Design review of the part built by this model. Coordinates are the model's own, in mm. Face numbers are marked on the shaded views. A direction names the side the tool comes from. Coordinates: 2 decimals unless noted, no trailing zeros. Write each loop counter-clockwise with the first axis right and the second up, starting at its lowest first coordinate (ties: lowest second). Pieces come first, ordered by that corner, then holes.
Q1. Take a section at A-A, the plane x = 62.5. Write out the cut boundary in (y, z), plus the area to 3 significant figures.
Q2. Take a section at C-C, the plane x = 99.5. Write out the cut boundary in (y, z).
Q3. For L1, parallel to Z at x = 62, y = 4; L2, parallel to X at y = 6, z = 50; L3, parallel to Z at x = 74, y = 45, list the stretches that pass through material, from the lowest coordinate up.
Q4. For the marked faces 1 and 2, list the 3-axis set-ups (+Z, -Z, +X, -X, +Y, -Y) from which the entire face can be reached by the end or side of a thin tool; tool diameter is ignored.
Q5. Take a section at B-B, the plane z = 50. Write out the cut boundary in (x, y), plus the area to 3 significant figures.
Q6. The part is to be moulded in two halves that separate along Z. For the marked faces 3, 4 and 5, say which applies: released by +Z, released by -Z, zero draft, split by the parting line, or undercut.
Q7. Take a section at D-D, the plane y = 26.5. Write out the cut boundary in (x, z), plus the area to 4 significant figures.
Q8. For pin 1 Ø8 at (x, z) = (36, 54) entering from +Y, flat-tipped, find the tip position at first contact; note if it passes through.
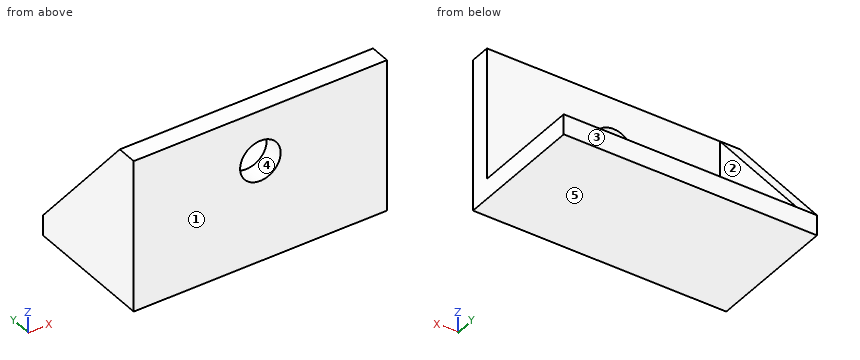
from build123d import *

# Parameters (mm, degrees)
BASE_PLATE_PROFILE_W  = 125
BASE_PLATE_PROFILE_H  = 10
BASE_PLATE_DEPTH      = 75
BACK_WALL_PROFILE_W   = 125
BACK_WALL_PROFILE_H   = 10
BACK_WALL_DEPTH       = 55
END_WALL_PROFILE_W    = 10
END_WALL_PROFILE_H    = 65
END_WALL_DEPTH        = 55
GUSSET_TRIM_CUT_DEPTH = 55
BASE_HOLE_20_SKETCH_R = 10
BASE_HOLE_20_DEPTH    = 55


with BuildPart() as part:
    # Base Plate Profile → Base Plate (new body)
    with BuildSketch(Plane.XY):
        with Locations((62.5, 5)):
            Rectangle(BASE_PLATE_PROFILE_W, BASE_PLATE_PROFILE_H)
    extrude(amount=BASE_PLATE_DEPTH)

    # Back Wall Profile → Back Wall (add)
    with BuildSketch(Plane(origin=(0, 10, 0), x_dir=(1, 0, 0), z_dir=(0, 1, 0))):
        with Locations((62.5, -5)):
            Rectangle(BACK_WALL_PROFILE_W, BACK_WALL_PROFILE_H)
    extrude(amount=BACK_WALL_DEPTH)

    # End Wall Profile → End Wall (add)
    with BuildSketch(Plane(origin=(0, 10, 0), x_dir=(1, 0, 0), z_dir=(0, 1, 0))):
        with Locations((5, -42.5)):
            Rectangle(END_WALL_PROFILE_W, END_WALL_PROFILE_H)
    extrude(amount=END_WALL_DEPTH)

    # Gusset Trim Profile → Gusset Trim Cut (cut)
    with BuildSketch(Plane(origin=(10, 0, 0), x_dir=(0, 0, -1), z_dir=(1, 0, 0))):
        Polygon((-10, 65), (-75, 10), (-75, 65), align=None)
    extrude(amount=-GUSSET_TRIM_CUT_DEPTH, mode=Mode.SUBTRACT)

    # Base Hole Ø20 Sketch → Base Hole Ø20 (cut)
    with BuildSketch(Plane(origin=(0, 10, 0), x_dir=(1, 0, 0), z_dir=(0, 1, 0))):
        with Locations(Location((62.5, -50, 0), (0, 0, 270))):
            Circle(BASE_HOLE_20_SKETCH_R)
    extrude(amount=-BASE_HOLE_20_DEPTH, mode=Mode.SUBTRACT)


solid = part.part
Responses:
1. outline: (0, 0) - (65, 0) - (65, 10) - (10, 10) - (10, 40) - (0, 40) - close; (0, 60) - (10, 60) - (10, 75) - (0, 75) - close
1. area: 1,100 mm2
2. outline: (0, 0) - (65, 0) - (65, 10) - (10, 10) - (10, 75) - (0, 75) - close
3. L1: z = 0 to 40.01, 59.99 to 75
3. L2: x = 0 to 52.5, 72.5 to 125
3. L3: z = 0 to 10
4. face 1: +Z, -Z, +X, -X, -Y
4. face 2: +Z, +X, +Y
5. outline: (0, 0) - (52.5, 0) - (52.5, 10) - (10, 10) - (10, 31.15) - (0, 31.15) - close; (72.5, 0) - (125, 0) - (125, 10) - (72.5, 10) - close
5. area: 1,260 mm2
6. face 3: zero draft
6. face 4: undercut
6. face 5: released by -Z
7. outline: (0, 0) - (125, 0) - (125, 10) - (10, 10) - (10, 55.5) - (0, 55.5) - close
7. area: 1,705 mm2
8. pin 1: stops at y = 10
